The listing builds one solid part. Answer for the finished solid, in the listing's coordinates (mm). Face numbers are marked on the shaded views. Coordinates: 2 decimals unless noted, no trailing zeros. Write each loop counter-clockwise with the first axis right and the second up, starting at its lowest first coordinate (ties: lowest second). Pieces come first, ordered by that corner, then holes. Notation, with made-up numbers: M 65,37 L 120,37 A26 cw 120,55 Z; hole C 24.5,80 d2. An arc over 180 degrees is marked long. Answer as CSV lines item,"result".
```python
from build123d import *

# Parameters (mm, degrees)
SKETCH_1_R      = 5.1
EXTRUDE_1_DEPTH = 3


with BuildPart() as part:
    # 草图1 → 凸台-拉伸1 (new, symmetric)
    with BuildSketch(Plane.XY):
        with BuildLine():
            Line((0, 14), (20, 14))
            Line((20, 14), (20, -14))
            Line((20, -14), (0, -14))
            ThreePointArc((0, -14), (-14, 0), (0, 14))
        make_face()
        Circle(SKETCH_1_R, mode=Mode.SUBTRACT)
    extrude(amount=EXTRUDE_1_DEPTH, both=True)


solid = part.part
```
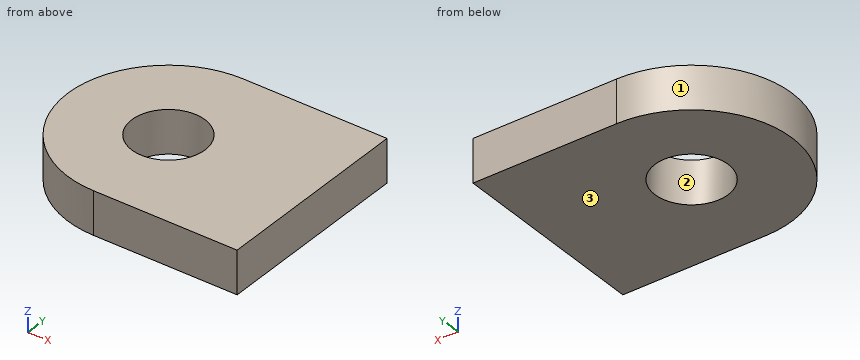
Q1. Find section C-C (x = -8.5). Give the vertices of the cut face in (y, z).
Output:
outline,"M -11.12,-3 L 11.12,-3 L 11.12,3 L -11.12,3 Z"
Q2. Find section B-B (z = -0.85). Give the vertices of the cut face in (x, y).
Output:
outline,"M 0,-14 L 20,-14 L 20,14 L 0,14 A14 ccw Z; hole C 0,0 d10.2"
Q3. Flat-ended cylindrical pins translate along their axes: pin 1 Ø3 at (x, z) = (-2.5, -1) entering from -Y; pin 2 Ø3 at (y, z) = (-11, 0.5) entering from -X. Find the tip coordinate at first contact, or state that the pin passes through.
Output:
pin 1,"y = -13.96"
pin 2,"x = -10.28"
Q4. Straight lines are drawn through the part: line 1 (Y direction, x = 0, z = 1.2); line 2 (X direction, y = -1.5, z = 2); line 3 (Y direction, x = 1, z = -2). For each, find the intervals that lie inside material, in ascending order.
Output:
line 1,"-14 to -5.1, 5.1 to 14"
line 2,"-13.92 to -4.87, 4.87 to 20"
line 3,"-14 to -5, 5 to 14"
Q5. Find section A-A (y = 0). Give the vertices of the cut face in (x, z).
Output:
outline,"M -14,-3 L -5.1,-3 L -5.1,3 L -14,3 Z; M 5.1,-3 L 20,-3 L 20,3 L 5.1,3 Z"
Q6. Find section D-D (y = -12). Give the vertices of the cut face in (x, z), and give its area (3 significant figures).
Output:
outline,"M -7.21,-3 L 20,-3 L 20,3 L -7.21,3 Z"
area,"163 mm2"
Q7. The mould has two halves that part along X. Classify the marked faces 1, 2 and 3: pulls with the +X half, pulls with the -X half, needs draft (parallel to the pull), parting line crosses it, or undercut.
Output:
face 1,"pulls with the -X half"
face 2,"undercut"
face 3,"needs draft"
